The listing builds one solid part. Answer for the finished solid, in the listing's coordinates (mm). A direction names the side the tool comes from. Round coordinates to 2 decimals unless told otherwise and drop trailing zeros. Order: outer loops, then holes, each group sorted by start corner. A loop starts at its lowest first (then second) coordinate and runs counter-clockwise, first axis right, second up. Notation, with made-up numbers: M 68,-39.75 L 87,-39.75 A29 cw 87,-7.75 Z; hole C 4,38 d9. An arc over 180 degrees is marked long. Put each result on its own line as item: value. Start each with the question number.
1. The part is cut by section B-B (x = 1). Give the vertices of the cut face in (y, z), then the cut area to 3 significant figures.
2. Consider line 1 (Y direction, x = 6.5, z = 0); line 2 (Y direction, x = 5.75, z = 1); line 3 (X direction, y = 8, z = 5.5). Determine where each line is inside the solid, lowest interval first.
3. Which of the six approach directions +Z, -Z, +X, -X, +Y, -Y give full straight-line access (tool end or side, diameter ignored) to faces 1 (the face through (5.94, -3.32, -0.74)), 2 (the face through (0, -4.3, 0.1)), 3 (the face through (10, -4, 0))?
4. The part is cut by section D-D (x = -12.75). Give the vertices of the cut face in (y, z).
5. The part is cut by section C-C (z = -8). Give the vertices of the cut face in (x, y).
6. The part is cut by section A-A (y = -6). Give the vertices of the cut face in (x, z), then the cut area to 3 significant figures.
7. Each of these flat-tipped pins is pushed along its axis until it touches: pin 1 Ø1 at (y, z) = (-6.5, -3) entering from -X; pin 2 Ø12 at (x, z) = (-4.5, 4.5) entering from +Y; pin 3 Ø2 at (x, z) = (0.5, 2.5) entering from -Y; pin 4 Ø6 at (x, y) = (-7, -7.5) entering from +Z. Where does it stop, or does it pass through?
from build123d import *

# Parameters (mm, degrees)
SKETCH_1_R             = 10
EXTRUDE_1_DEPTH        = 10
SKETCH_2_R             = 4
EXTRUDE_2_DEPTH        = 15
HOLE_WIZARD_M8_1_D     = 6.8
HOLE_WIZARD_M8_1_DEPTH = 8
HOLE_WIZARD_M8_1_TIP   = 2.042926105


with BuildPart() as part:
    # 草图1 → 凸台-拉伸1 (new body)
    with BuildSketch(Plane(origin=(0, 0, 0), x_dir=(0, 0, -1), z_dir=(1, 0, 0))):
        Circle(SKETCH_1_R)
    extrude(amount=EXTRUDE_1_DEPTH)

    # 草图2 → 凸台-拉伸2 (add)
    with BuildSketch(Plane.ZY):
        Circle(SKETCH_2_R)
    extrude(amount=EXTRUDE_2_DEPTH)

    # M8 螺纹孔1
    with Locations(Plane(origin=(10, 0, 0), x_dir=(0, 0, -1), z_dir=(1, 0, 0))):
        with Locations((0, 0)):
            Hole(HOLE_WIZARD_M8_1_D / 2, depth=HOLE_WIZARD_M8_1_DEPTH)
            with Locations((0, 0, -(HOLE_WIZARD_M8_1_DEPTH + HOLE_WIZARD_M8_1_TIP / 2))):  # 118° drill point
                Cone(0, HOLE_WIZARD_M8_1_D / 2, HOLE_WIZARD_M8_1_TIP, mode=Mode.SUBTRACT)


solid = part.part
Resolved:
1. outline: C 0,0 d20; hole C 0,0 d3.47
1. area: 305 mm2
2. line 1: -10 to -3.4, 3.4 to 10
2. line 2: -9.95 to -3.25, 3.25 to 9.95
2. line 3: 0 to 10
3. face 1: +X
3. face 2: -X
3. face 3: +Z, -Z, +X, +Y, -Y
4. outline: C 0,0 d8
5. outline: M 0,-6 L 10,-6 L 10,6 L 0,6 Z
6. outline: M 0,-8 L 10,-8 L 10,8 L 0,8 Z
6. area: 160 mm2
7. pin 1: x = 0
7. pin 2: y = 9.99
7. pin 3: y = -9.89
7. pin 4: through
